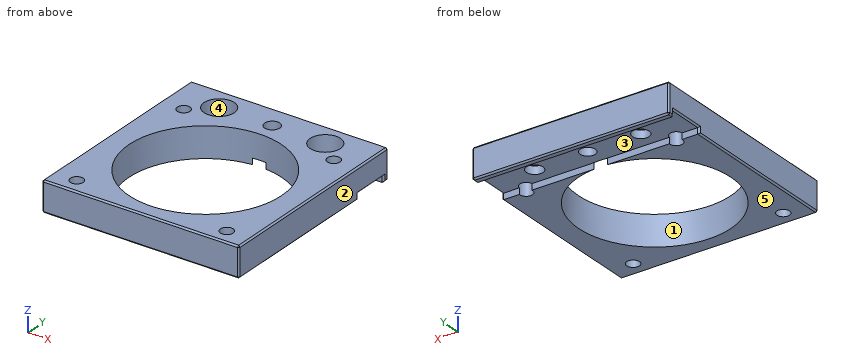
```python
from build123d import *

# Parameters (mm, degrees)
SKETCH_1_W                     = 65
SKETCH_1_H                     = 69
EXTRUDE_1_DEPTH                = 10
SKETCH_2_W                     = 2
SKETCH_2_H                     = 12
CUT_EXTRUDE_1_DEPTH            = 75.264729179
SKETCH_3_R                     = 25.1
CUT_EXTRUDE_2_DEPTH            = 49.440685379
HOLE_WIZARD_M5_1_D             = 4.2
HOLE_WIZARD_M5_1_2_D           = 5.5
HOLE_WIZARD_M5_1_2_CBORE_D     = 10
HOLE_WIZARD_M5_1_2_CBORE_DEPTH = 5.4
MM_1_D                         = 5
CHAMFER_1_SIZE                 = 0.5


with BuildPart() as part:
    # 草图1 → 凸台-拉伸1 (new body)
    with BuildSketch(Plane.XY):
        Rectangle(SKETCH_1_W, SKETCH_1_H)
    extrude(amount=EXTRUDE_1_DEPTH)

    # 草图2 → 切除-拉伸1 (cut, through all)
    with BuildSketch(Plane.ZY.offset(32.5)):
        with Locations((1, 26.5)):
            Rectangle(SKETCH_2_W, SKETCH_2_H)
    extrude(amount=-CUT_EXTRUDE_1_DEPTH, mode=Mode.SUBTRACT)

    # 草图3 → 切除-拉伸2 (cut, through all)
    with BuildSketch(Plane.XY.offset(10)):
        with Locations((0, -4.5)):
            Circle(SKETCH_3_R)
    extrude(amount=-CUT_EXTRUDE_2_DEPTH, mode=Mode.SUBTRACT)

    # Hole Wizard M5 _1 (through all)
    with Locations(Plane.XY.offset(10)):
        with Locations((24.748737342, 20.248737342), (24.748737342, -29.248737342), (-24.748737342, -29.248737342), (-24.748737342, 20.248737342)):
            Hole(HOLE_WIZARD_M5_1_D / 2)

    # Hole Wizard M5 _1 2 (through all)
    with Locations(Plane.XY.offset(10)):
        with Locations((17.5, 26.5), (-17.5, 26.5)):
            CounterBoreHole(HOLE_WIZARD_M5_1_2_D / 2, HOLE_WIZARD_M5_1_2_CBORE_D / 2, HOLE_WIZARD_M5_1_2_CBORE_DEPTH)

    # 大小mm 暗销孔1 (through all)
    with Locations(Plane.XY.offset(10)):
        with Locations((0, 26.5)):
            Hole(MM_1_D / 2)

    # 倒角1
    chamfer_1_edges = [part.edges().sort_by_distance(p)[0] for p in [
        (-32.5, 0, 10),
        (32.5, 33.5, 0),
        (-32.5, -7, 0),
        (0, -34.5, 10),
        (32.5, 32.5, 1),
        (32.5, 26.5, 2),
        (32.5, 20.5, 1),
        (-32.5, 20.5, 1),
        (-32.5, 26.5, 2),
        (-32.5, 32.5, 1),
        (32.5, 0, 10),
        (0, -34.5, 0),
        (-32.5, 33.5, 0),
        (0, 34.5, 0),
        (32.5, -7, 0),
        (32.5, -34.5, 5),
        (-32.5, -34.5, 5),
        (-32.5, 34.5, 5),
        (32.5, 34.5, 5),
        (0, 34.5, 10),
    ]]
    chamfer(chamfer_1_edges, length=CHAMFER_1_SIZE)


solid = part.part
```
Source: CAD feature listing. Evaluate the final solid. Frame: model axes, mm. Face numbers are marked on the shaded views. A direction names the side the tool comes from. Coordinates: 2 decimals unless noted, no trailing zeros. Loops run counter-clockwise (first coordinate to the right, second up) from the corner with the lowest first, then second, coordinate; pieces in that order, holes last. Notation, with made-up numbers: M 41,84 L 60,84 A27 ccw 60,119 Z; hole C 6,62 d4. An arc over 180 degrees is marked long. Use CSV: the item, a comma, the result in double quotes.
(1) Cut plane C-C on z = 8.5. Give the number of separate pieces and of enclosed holes in the cut face, and give its area (3 significant figures).
Answers follow:
separate pieces,"1"
enclosed holes,"8"
area,"2,270 mm²"
(2) Draft query along X for the marked faces 1, 2 and 3. Return one class per face: pulls with the +X half, pulls with the -X half, needs draft (parallel to the pull), parting line crosses it, or undercut.
Answers follow:
face 1,"undercut"
face 2,"pulls with the +X half"
face 3,"needs draft"
(3) Line query: line 1 (Y direction, x = 0, z = 8.75); line 2 (X direction, y = -4.5, z = 5.5); line 3 (Y direction, x = 0.5, z = 8.25). Output: solid intervals per line, ascending. Write a range as [from, to].
Answers follow:
line 1,"[-34.5, -29.6], [20.6, 24], [29, 34.5]"
line 2,"[-32.5, -25.1], [25.1, 32.5]"
line 3,"[-34.5, -29.6], [20.6, 24.05], [28.95, 34.5]"
(4) Cut plane D-D on y = 26.5. Return loops of the section in (x, z), and give its area (3 significant figures).
Answers follow:
outline,"M -32.5,2.5 L -32,2 L -20.25,2 L -20.25,4.6 L -22.5,4.6 L -22.5,10 L -32,10 L -32.5,9.5 Z; M -14.75,2 L -2.5,2 L -2.5,10 L -12.5,10 L -12.5,4.6 L -14.75,4.6 Z; M 2.5,2 L 14.75,2 L 14.75,4.6 L 12.5,4.6 L 12.5,10 L 2.5,10 Z; M 20.25,2 L 32,2 L 32.5,2.5 L 32.5,9.5 L 32,10 L 22.5,10 L 22.5,4.6 L 20.25,4.6 Z"
area,"343 mm²"
(5) Cut plane A-A on x = 0. Return loops of the section in (y, z).
Answers follow:
outline,"M -34.5,0.5 L -34,0 L -29.6,0 L -29.6,10 L -34,10 L -34.5,9.5 Z; M 20.6,2 L 24,2 L 24,10 L 20.6,10 Z; M 29,2 L 32.5,2 L 32.5,0 L 34,0 L 34.5,0.5 L 34.5,9.5 L 34,10 L 29,10 Z"
(6) Cut plane B-B on y = -4.5. Return loops of the section in (x, z), and give its area (4 significant figures).
Answers follow:
outline,"M -32.5,0.5 L -32,0 L -25.1,0 L -25.1,10 L -32,10 L -32.5,9.5 Z; M 25.1,0 L 32,0 L 32.5,0.5 L 32.5,9.5 L 32,10 L 25.1,10 Z"
area,"147.5 mm²"
(7) Contact query for a flat-ended pin moving along its axis: pin 1 (9 mm diameter, centred on x = -17.5, y = 26.5, fed in from +Z). Output: stop coordinate, or through.
Answers follow:
pin 1,"z = 4.6"
(8) Reachability of the marked faces 4 and 5 from +Z, -Z, +X, -X, +Y, -Y: full face, straight path, thin tool, end or side. Return the list, or none.
Answers follow:
face 4,"+Z"
face 5,"-Z, +X, -X, +Y, -Y"
